```python
from build123d import *

# Parameters (mm, degrees)
SKETCH4_W               = 100
SKETCH4_H               = 100
SKETCH4_W_2             = 81
SKETCH4_H_2             = 81
BOSS_EXTRUDE1_DEPTH     = 40
SKETCH5_R               = 87.5
BOSS_EXTRUDE2_DEPTH     = 10
SKETCH6_OUTSIDE_W       = 227.498
SKETCH6_OUTSIDE_H       = 227.498
SKETCH6_OUTSIDE_W_2     = 100
SKETCH6_OUTSIDE_H_2     = 212.75110477
CUT_EXTRUDE1_DEPTH      = 10
SKETCH7_W               = 81
SKETCH7_H               = 81
CUT_EXTRUDE2_DEPTH      = 10
SKETCH8_R               = 4.5
CUT_EXTRUDE3_DEPTH      = 10
M16_TAPPED_HOLE1_D      = 14
M16_TAPPED_HOLE2_D      = 14
SIZE_MM_DOWEL_HOLE2_D   = 8
MM_2_D                  = 8
RIB2_REACH              = 120.98
SKETCH18_WALL_W         = 284.681440236
SKETCH18_WALL_H         = 5
MIRROR2_COPY_1_REACH    = 120.98
MIRROR2_COPY_1_SKETCH_W = 284.681440236
MIRROR2_COPY_1_SKETCH_H = 5


with BuildPart() as part:
    # Sketch4 → Boss-Extrude1 (new body)
    with BuildSketch(Plane(origin=(0, 0, 0), x_dir=(0, 0, -1), z_dir=(1, 0, 0))):
        Rectangle(SKETCH4_W, SKETCH4_H)
        Rectangle(SKETCH4_W_2, SKETCH4_H_2, mode=Mode.SUBTRACT)
    extrude(amount=BOSS_EXTRUDE1_DEPTH)

    # Sketch5 → Boss-Extrude2 (add)
    with BuildSketch(Plane.ZY):
        Circle(SKETCH5_R)
    extrude(amount=BOSS_EXTRUDE2_DEPTH)

    # Sketch6 outside → Cut-Extrude1 (cut)
    with BuildSketch(Plane.ZY.offset(10)):
        Rectangle(SKETCH6_OUTSIDE_W, SKETCH6_OUTSIDE_H)
        Rectangle(SKETCH6_OUTSIDE_W_2, SKETCH6_OUTSIDE_H_2, mode=Mode.SUBTRACT)
    extrude(amount=-CUT_EXTRUDE1_DEPTH, mode=Mode.SUBTRACT)

    # Sketch7 → Cut-Extrude2 (cut)
    with BuildSketch(Plane(origin=(0, 0, 0), x_dir=(0, 0, -1), z_dir=(1, 0, 0))):
        Rectangle(SKETCH7_W, SKETCH7_H)
    extrude(amount=-CUT_EXTRUDE2_DEPTH, mode=Mode.SUBTRACT)

    # Sketch8 → Cut-Extrude3 (cut)
    with BuildSketch(Plane(origin=(0, 0, 0), x_dir=(0, 0, -1), z_dir=(1, 0, 0))):
        with Locations((-36.25, 62.786841774)):
            Circle(SKETCH8_R)
        with Locations((0, 72.5)):
            Circle(SKETCH8_R)
        with Locations((36.25, 62.786841774)):
            Circle(SKETCH8_R)
        with Locations(Location((36.25, -62.786841774, 0), (0, 0, 180))):
            Circle(SKETCH8_R)
        with Locations(Location((0, -72.5, 0), (0, 0, 180))):
            Circle(SKETCH8_R)
        with Locations(Location((-36.25, -62.786841774, 0), (0, 0, 180))):
            Circle(SKETCH8_R)
    extrude(amount=-CUT_EXTRUDE3_DEPTH, mode=Mode.SUBTRACT)

    # M16 Tapped Hole1 (through all)
    with Locations(Plane.XY.offset(50)):
        with Locations((26, 0)):
            Hole(M16_TAPPED_HOLE1_D / 2)

    # M16 Tapped Hole2 (through all)
    with Locations(Plane(origin=(0, 50, 0), x_dir=(1, 0, 0), z_dir=(0, 1, 0))):
        with Locations((26, 0)):
            Hole(M16_TAPPED_HOLE2_D / 2)

    # Size mm Dowel Hole2 (through all)
    with Locations(Plane.XY.offset(50)):
        with Locations((7, 0)):
            Hole(SIZE_MM_DOWEL_HOLE2_D / 2)

    # 大小mm 暗销孔2 (through all)
    with Locations(Plane(origin=(0, 50, 0), x_dir=(1, 0, 0), z_dir=(0, 1, 0))):
        with Locations((7, 0)):
            Hole(MM_2_D / 2)

    # Sketch18 wall → Rib2 (add, up to next)
    with BuildSketch(Plane(origin=(20, 60, 20), x_dir=(-0.894427191, 0.4472135955, 0), z_dir=(-0.4472135955, -0.894427191, 0)), mode=Mode.PRIVATE) as rib2_sk1:
        Rectangle(SKETCH18_WALL_W, SKETCH18_WALL_H)
    rib2_tool1 = extrude(rib2_sk1.sketch, amount=RIB2_REACH, mode=Mode.PRIVATE) - part.part
    rib2 = rib2_tool1.solids().sort_by_distance((20, 60, 20))[0]
    add(rib2)

    # Mirror1: Rib2 across plane
    add(rib2.mirror(Plane.ZX))

    # Mirror2: Rib2 across plane
    add(rib2.mirror(Plane.XY))

    # Mirror2 copy 1 sketch → Mirror2 copy 1 (add, up to next)
    with BuildSketch(Plane(origin=(20, -60, -20), x_dir=(-0.894427191, -0.4472135955, 0), z_dir=(-0.4472135955, 0.894427191, 0)), mode=Mode.PRIVATE) as mirror2_copy_1_sk1:
        Rectangle(MIRROR2_COPY_1_SKETCH_W, MIRROR2_COPY_1_SKETCH_H)
    mirror2_copy_1_tool1 = extrude(mirror2_copy_1_sk1.sketch, amount=MIRROR2_COPY_1_REACH, mode=Mode.PRIVATE) - part.part
    add(mirror2_copy_1_tool1.solids().sort_by_distance((20, -60, -20))[0])


solid = part.part
```
Input: part model. Units: mm. Frame: model coordinates. A direction names the side the tool comes from. Give positions to 0.01 mm unless a question says otherwise; leave off trailing zeros. Write each loop counter-clockwise with the first axis right and the second up, starting at its lowest first coordinate (ties: lowest second). Pieces come first, ordered by that corner, then holes. Notation, with made-up numbers: (-29, 88.5) - (5, 88.5) arc R24 ccw to (5, 115.5) - close; hole circle Ø5 at (7, 34.5). An arc over 180 degrees is marked (long way). Write item = value, one per line. Start each with the question number.
1. Section query C-C, the plane z = 36.25. Output: boundary loops of the cut face in (x, y), then the cut area to 3 significant figures.
2. Access query for faces 1 (the flat face through (20, -50, 4)), 2 (the flat face through (20, 50, -36)), 3 (the flat face through (14, -58, -22.5)). Directions: +Z, -Z, +X, -X, +Y, -Y. A direction counts if a zero-diameter tool reaches every point of the face in a straight line with its end or side. Return the directions, or none.
3. First-contact query: pin 1 Ø16 at (x, z) = (26, 0) entering from -Y; pin 2 Ø16 at (x, y) = (19.5, 62) entering from +Z; pin 3 Ø19 at (y, z) = (63, 4) entering from +X; pin 4 Ø22 at (x, y) = (16, 59.5) entering from -Z. Flat tips, straight axial feed; report the tip coordinate or a pass-through.
4. Ray query, L1, parallel to Z at x = 26, y = 47; L2, parallel to Y at x = 7, z = 44; L3, parallel to Z at x = 36.5, y = 32.5. Return the intervals inside material, ascending.
5. Mould query, pull axis Z, two halves, no side actions, for faces 4 (the flat face through (14, 58, -22.5)), 5 (the cylindrical face through (-4.93, -87.497, -0.745)), 6 (the flat face through (20, 50, 4)). Classes: released by +Z, released by -Z, zero draft, split by the parting line, or undercut.
6. Section query B-B, the plane y = 0. Output: boundary loops of the cut face in (x, z), then the cut area to 3 significant figures.
7. Section query A-A, the plane x = 17. Output: boundary loops of the cut face in (y, z).
8. Section query D-D, the plane y = -35. Output: boundary loops of the cut face in (x, z), then the cut area to 3 significant figures.
Check sheet entries:
q1.outline = (-10, -79.64) - (0, -79.64) - (0, -67.29) - (-10, -67.29) - close; (-10, -58.29) - (0, -58.29) - (0, -50) - (40, -50) - (40, -40.5) - (-10, -40.5) - close; (-10, 40.5) - (40, 40.5) - (40, 50) - (0, 50) - (0, 58.29) - (-10, 58.29) - close; (-10, 67.29) - (0, 67.29) - (0, 79.64) - (-10, 79.64) - close
q1.area = 1,360 mm2
q2.face_1 = +X, -Y
q2.face_2 = -Z, +X, +Y
q2.face_3 = -Z, +X, -Y
q3.pin_1 = -50
q3.pin_2 = 22.5
q3.pin_3 = 0
q3.pin_4 = -50
q4.L1 = -50 to -7, 7 to 50
q4.L2 = -50 to -4, 4 to 50
q4.L3 = -50 to -40.5, 40.5 to 50
q5.face_4 = released by -Z
q5.face_5 = split by the parting line
q5.face_6 = undercut
q6.outline = (-10, -50) - (3, -50) - (3, -40.5) - (-10, -40.5) - close; (-10, 40.5) - (3, 40.5) - (3, 50) - (-10, 50) - close; (11, -50) - (19, -50) - (19, -40.5) - (11, -40.5) - close; (11, 40.5) - (19, 40.5) - (19, 50) - (11, 50) - close; (33, -50) - (40, -50) - (40, -40.5) - (33, -40.5) - close; (33, 40.5) - (40, 40.5) - (40, 50) - (33, 50) - close
q6.area = 532 mm2
q7.outline = (-61.5, -22.5) - (-50, -22.5) - (-50, -50) - (50, -50) - (50, -22.5) - (61.5, -22.5) - (61.5, -17.5) - (50, -17.5) - (50, 17.5) - (61.5, 17.5) - (61.5, 22.5) - (50, 22.5) - (50, 50) - (-50, 50) - (-50, 22.5) - (-61.5, 22.5) - (-61.5, 17.5) - (-50, 17.5) - (-50, -17.5) - (-61.5, -17.5) - close; hole (-40.5, -40.5) - (40.5, -40.5) - (40.5, 40.5) - (-40.5, 40.5) - close
q8.outline = (-10, -50) - (40, -50) - (40, -40.5) - (-10, -40.5) - close; (-10, 40.5) - (40, 40.5) - (40, 50) - (-10, 50) - close
q8.area = 950 mm2
